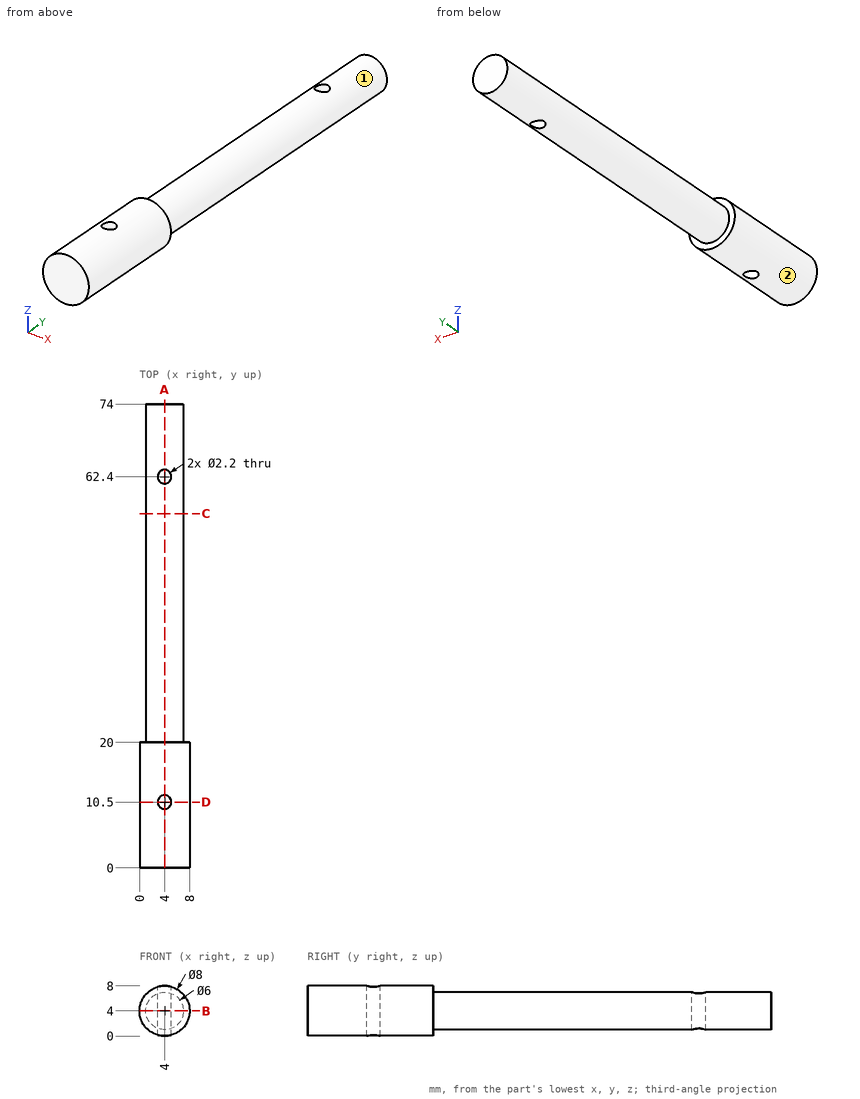
Part print with two shaded views. Sizes in mm from the minimum x, y, z corner. A direction names the side the tool comes from. Round coordinates to 2 decimals unless told otherwise and drop trailing zeros. Write each loop counter-clockwise with the first axis right and the second up, starting at its lowest first coordinate (ties: lowest second). Pieces come first, ordered by that corner, then holes. Notation, with made-up numbers: M 1,61 L 13,61 A19 ccw 13,90 Z; hole C 30.25,20.25 d7. An arc over 180 degrees is marked long. Answer as CSV lines item,"result". Start each with the question number.
1) Which spindle directions (+Z, -Z, +X, -X, +Y, -Y) get a long thin tool onto all of the face, cutting with end or side? Do the marked faces 1 and 2. Say none if no direction does.
2) Band-saw the part on B-B (z = 4). List the corners of the cut face in (x, y), then the cut area to 3 significant figures.
3) Drop flat-ended pins along their axis: pin 1 (4 mm diameter, centred on y = 25.5, z = 5, fed in from +X); pin 2 (2 mm diameter, centred on y = 60.5, z = 6.5, fed in from -X); pin 3 (2.5 mm diameter, centred on x = 4, y = 62.4, fed in from -Z). Give the stop position or say it passes through.
4) Band-saw the part on A-A (x = 4). List the corners of the cut face in (y, z), then the cut area to 3 significant figures.
5) Band-saw the part on C-C (y = 56.5). List the corners of the cut face in (x, z), then the cut area to 3 significant figures.
6) Band-saw the part on D-D (y = 10.5). List the corners of the cut face in (x, z), then the cut area to 3 significant figures.
7) Drill centre lines: L1, parallel to Y at x = 4, z = 3.25; L2, parallel to Z at x = 3.75, y = 60; L3, parallel to Y at x = 1.75, z = 7.25. Where is each one in solid material? Low to high.
Worked out:
1,face 1,"+Y"
1,face 2,"+Y, -Y"
2,outline,"M 0,0 L 8,0 L 8,20 L 7,20 L 7,74 L 1,74 L 1,20 L 0,20 Z; hole C 4,10.5 d2.2; hole C 4,62.4 d2.2"
2,area,"476 mm²"
3,pin 1,"x = 7"
3,pin 2,"x = 1.4"
3,pin 3,"z = 1"
4,outline,"M 0,0 L 9.4,0 L 9.4,8 L 0,8 Z; M 11.6,0 L 20,0 L 20,1 L 61.3,1 L 61.3,7 L 20,7 L 20,8 L 11.6,8 Z; M 63.5,1 L 74,1 L 74,7 L 63.5,7 Z"
4,area,"453 mm²"
5,outline,"C 4,4 d6"
5,area,"28.3 mm²"
6,outline,"M 2.9,0.15 L 2.9,7.85 A4 ccw Z; M 5.1,0.15 A4 ccw 5.1,7.85 Z"
6,area,"32.9 mm²"
7,L1,"0 to 9.4, 11.6 to 61.3, 63.5 to 74"
7,L2,"1.01 to 6.99"
7,L3,"0 to 20"
